from build123d import *

# Parameters (mm, degrees)
SKETCH1_W           = 445
SKETCH1_H           = 100
SKETCH1_R           = 9
BOSS_EXTRUDE1_DEPTH = 20


with BuildPart() as part:
    # Sketch1 → Boss-Extrude1 (new body)
    with BuildSketch(Plane.XY):
        with Locations((222.5, 50)):
            Rectangle(SKETCH1_W, SKETCH1_H)
        with Locations((15, 50)):
            Circle(SKETCH1_R, mode=Mode.SUBTRACT)
        with Locations(Location((430, 50, 0), (0, 0, 180))):
            Circle(SKETCH1_R, mode=Mode.SUBTRACT)
    extrude(amount=BOSS_EXTRUDE1_DEPTH)


solid = part.part
Here's how the part is built. I have some questions about the finished solid (model axes, mm). Round coordinates to 2 decimals unless told otherwise and drop trailing zeros. Order: outer loops, then holes, each group sorted by start corner. A loop starts at its lowest first (then second) coordinate and runs counter-clockwise, first axis right, second up. Notation, with made-up numbers: (50, 21.25) -> (87, 21.25) arc R23 cw to (87, 30.25) -> close; hole circle Ø9 at (57.5, 66.25). An arc over 180 degrees is marked (long way). Return JSON: item names as keys, results as strings.
Q1. If we section it at B-B on y = 50: List the corners of the cut face in (x, z) for me, plus the area to 3 significant figures.
Filled sheet:
{"outline": "(0, 0) -> (6, 0) -> (6, 20) -> (0, 20) -> close; (24, 0) -> (421, 0) -> (421, 20) -> (24, 20) -> close; (439, 0) -> (445, 0) -> (445, 20) -> (439, 20) -> close", "area": "8,180 mm^2"}
Q2. If we section it at A-A on x = 15: List the corners of the cut face in (y, z) for me, plus the area to 3 significant figures.
Filled sheet:
{"outline": "(0, 0) -> (41, 0) -> (41, 20) -> (0, 20) -> close; (59, 0) -> (100, 0) -> (100, 20) -> (59, 20) -> close", "area": "1,640 mm^2"}
Q3. I need wall thicknesses on line 1 along Y through (x, z) = (430, 5); line 2 along X through (y, z) = (56, 18.75). Which ranges of each line are inside material? Lowest first, please. Write a range as from..to.
Filled sheet:
{"line 1": "y = 0..41, 59..100", "line 2": "x = 0..8.29, 21.71..423.29, 436.71..445"}
Q4. If we mould it in two halves opening along X, with no side actions, what happens to faces 1 (the flat face through (445, 49, 10)), 2 (the flat face through (0, 49, 10)), 3 (the flat face through (219, 51, 0)), 4 (the cylindrical face through (421.416, 47.297, 9.86))? For each: released by +X, released by -X, zero draft, split by the parting line, or undercut.
Filled sheet:
{"face 1": "released by +X", "face 2": "released by -X", "face 3": "zero draft", "face 4": "undercut"}
